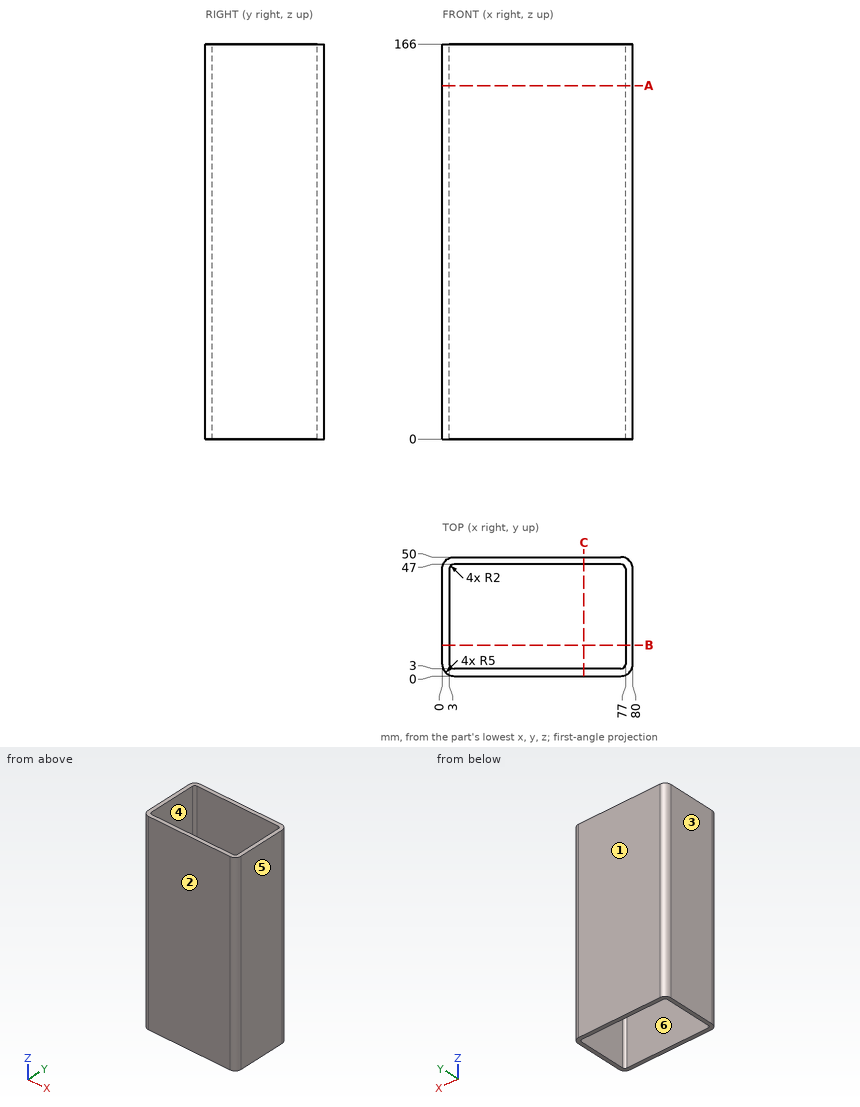
Design review of the part shown in the three views and the two pictorial views. Dimensions are in mm from the part's minimum x, y and z. A direction names the side the tool comes from. Round coordinates to 2 decimals unless told otherwise and drop trailing zeros. Write each loop counter-clockwise with the first axis right and the second up, starting at its lowest first coordinate (ties: lowest second). Pieces come first, ordered by that corner, then holes. Notation, with made-up numbers: (-37, 38) -> (-3, 38) arc R21 ccw to (-3, 62) -> close; hole circle Ø6 at (48.25, -29). An arc over 180 degrees is marked (long way). Use one line per item in the form item = value.
1) To check wall thickness, follow L1, parallel to X at y = 5.5, z = 106.5; L2, parallel to Y at x = 55.5, z = 45; L3, parallel to X at y = 45.5, z = 46. State the ranges of each line that lie inside material, in increasing order. Write a range as from..to.
Found:
L1 = 0..3, 77..80
L2 = 0..3, 47..50
L3 = 0.03..3.06, 76.94..79.97
2) Mouldability with a two-part tool opening along Y and no side actions: class the marked faces 1, 2, 3 and 4 as +Y half, -Y half, draft (parallel to the pull), parting line (faces both ways), or undercut.
Found:
face_1 = +Y half
face_2 = -Y half
face_3 = draft
face_4 = undercut
3) Tool access review of the marked faces 5 and 6: name each direction out of +Z, -Z, +X, -X, +Y, -Y from which nothing blocks a thin tool from reaching the whole face with its end or side.
Found:
face_5 = +Z, -Z, +X, +Y, -Y
face_6 = +Z, -Z
4) Take a section at C-C, the plane x = 59.5. Write out the cut boundary in (y, z), and give its area (3 significant figures).
Found:
outline = (0, 0) -> (3, 0) -> (3, 166) -> (0, 166) -> close; (47, 0) -> (50, 0) -> (50, 166) -> (47, 166) -> close
area = 996 mm2
5) Take a section at A-A, the plane z = 148.5. Write out the cut boundary in (x, y), and give its area (3 significant figures).
Found:
outline = (0, 5) arc R5 ccw to (5, 0) -> (75, 0) arc R5 ccw to (80, 5) -> (80, 45) arc R5 ccw to (75, 50) -> (5, 50) arc R5 ccw to (0, 45) -> close; hole (3, 5) arc R2 ccw to (5, 3) -> (75, 3) arc R2 ccw to (77, 5) -> (77, 45) arc R2 ccw to (75, 47) -> (5, 47) arc R2 ccw to (3, 45) -> close
area = 726 mm2
6) Clearance check with a flat-ended pin moving along its axis: pin 1 (1 mm diameter, centred on x = 70, z = 58.5, fed in from -Y). State where the tip first meets the part, or that it passes through.
Found:
pin_1 = 0
7) Take a section at B-B, the plane y = 13. Write out the cut boundary in (x, z).
Found:
outline = (0, 0) -> (3, 0) -> (3, 166) -> (0, 166) -> close; (77, 0) -> (80, 0) -> (80, 166) -> (77, 166) -> close
